from build123d import *

# Parameters (mm, degrees)
BOSS_EXTRUDE1_DEPTH             = 245
SKETCH6_R                       = 23.25
CUT_EXTRUDE1_DEPTH              = 3
F_6_5_6_5_DIAMETER_HOLE1_D      = 6.5
F_12_0_12_DIAMETER_HOLE1_REACH  = 253.446
F_12_0_12_DIAMETER_HOLE1_BORE_R = 6
M4_TAPPED_HOLE1_REACH           = 253.446
M4_TAPPED_HOLE1_BORE_R          = 1.65
CUT_EXTRUDE2_DEPTH              = 259.505319094
SKETCH12_R                      = 5
BOSS_EXTRUDE2_DEPTH             = 3
M5_TAPPED_HOLE1_D               = 4.2
M3_TAPPED_HOLE1_D               = 2.5
M3_TAPPED_HOLE1_DEPTH           = 3
CUT_EXTRUDE3_REACH              = 253.446
SKETCH17_R                      = 4


with BuildPart() as part:
    # Sketch1 → Boss-Extrude1 (new body)
    with BuildSketch(Plane.XY):
        with BuildLine():
            Line((-35, 20), (35, 20))
            ThreePointArc((35, 20), (38.535533906, 18.535533906), (40, 15))
            Line((40, 15), (40, -15))
            ThreePointArc((40, -15), (38.535533906, -18.535533906), (35, -20))
            Line((35, -20), (-35, -20))
            ThreePointArc((-35, -20), (-38.535533906, -18.535533906), (-40, -15))
            Line((-40, -15), (-40, 15))
            ThreePointArc((-40, 15), (-38.535533906, 18.535533906), (-35, 20))
        make_face()
        with BuildLine():
            Line((-37, 15), (-37, -15))
            ThreePointArc((-37, -15), (-36.414213562, -16.414213562), (-35, -17))
            Line((-35, -17), (35, -17))
            ThreePointArc((35, -17), (36.414213562, -16.414213562), (37, -15))
            Line((37, -15), (37, 15))
            ThreePointArc((37, 15), (36.414213562, 16.414213562), (35, 17))
            Line((35, 17), (-35, 17))
            ThreePointArc((-35, 17), (-36.414213562, 16.414213562), (-37, 15))
        make_face(mode=Mode.SUBTRACT)
    extrude(amount=BOSS_EXTRUDE1_DEPTH)

    # Sketch6 → Cut-Extrude1 (cut)
    with BuildSketch(Plane.XZ.offset(20)):
        with Locations(Location((0, 42, 0), (0, 0, 270))):
            Circle(SKETCH6_R)
    extrude(amount=-CUT_EXTRUDE1_DEPTH, mode=Mode.SUBTRACT)

    # Ø6.5 (6.5) Diameter Hole1 (through all)
    with Locations(Plane(origin=(0, 20, 0), x_dir=(1, 0, 0), z_dir=(0, 1, 0))):
        with Locations((-25, -17), (25, -17), (25, -67), (-25, -67)):
            Hole(F_6_5_6_5_DIAMETER_HOLE1_D / 2)

    # Ø12.0 (12) Diameter Hole1 bore → Ø12.0 (12) Diameter Hole1 (cut, up to next)
    with BuildSketch(Plane(origin=(0, 20, 0), x_dir=(1, 0, 0), z_dir=(0, 1, 0)), mode=Mode.PRIVATE) as f_12_0_12_diameter_hole1_sk1:
        with Locations((-25, -17)):
            Circle(F_12_0_12_DIAMETER_HOLE1_BORE_R)
    f_12_0_12_diameter_hole1_tool1 = extrude(f_12_0_12_diameter_hole1_sk1.sketch, amount=-F_12_0_12_DIAMETER_HOLE1_REACH, mode=Mode.PRIVATE) & part.part
    # Ø12.0 (12) Diameter Hole1 bore → Ø12.0 (12) Diameter Hole1 (cut, up to next)
    with BuildSketch(Plane(origin=(0, 20, 0), x_dir=(1, 0, 0), z_dir=(0, 1, 0)), mode=Mode.PRIVATE) as f_12_0_12_diameter_hole1_sk2:
        with Locations((25, -17)):
            Circle(F_12_0_12_DIAMETER_HOLE1_BORE_R)
    f_12_0_12_diameter_hole1_tool2 = extrude(f_12_0_12_diameter_hole1_sk2.sketch, amount=-F_12_0_12_DIAMETER_HOLE1_REACH, mode=Mode.PRIVATE) & part.part
    # Ø12.0 (12) Diameter Hole1 bore → Ø12.0 (12) Diameter Hole1 (cut, up to next)
    with BuildSketch(Plane(origin=(0, 20, 0), x_dir=(1, 0, 0), z_dir=(0, 1, 0)), mode=Mode.PRIVATE) as f_12_0_12_diameter_hole1_sk3:
        with Locations((25, -67)):
            Circle(F_12_0_12_DIAMETER_HOLE1_BORE_R)
    f_12_0_12_diameter_hole1_tool3 = extrude(f_12_0_12_diameter_hole1_sk3.sketch, amount=-F_12_0_12_DIAMETER_HOLE1_REACH, mode=Mode.PRIVATE) & part.part
    # Ø12.0 (12) Diameter Hole1 bore → Ø12.0 (12) Diameter Hole1 (cut, up to next)
    with BuildSketch(Plane(origin=(0, 20, 0), x_dir=(1, 0, 0), z_dir=(0, 1, 0)), mode=Mode.PRIVATE) as f_12_0_12_diameter_hole1_sk4:
        with Locations((-25, -67)):
            Circle(F_12_0_12_DIAMETER_HOLE1_BORE_R)
    f_12_0_12_diameter_hole1_tool4 = extrude(f_12_0_12_diameter_hole1_sk4.sketch, amount=-F_12_0_12_DIAMETER_HOLE1_REACH, mode=Mode.PRIVATE) & part.part
    add(f_12_0_12_diameter_hole1_tool1.solids().sort_by_distance((-25, 20, 17))[0], mode=Mode.SUBTRACT)
    add(f_12_0_12_diameter_hole1_tool2.solids().sort_by_distance((25, 20, 17))[0], mode=Mode.SUBTRACT)
    add(f_12_0_12_diameter_hole1_tool3.solids().sort_by_distance((25, 20, 67))[0], mode=Mode.SUBTRACT)
    add(f_12_0_12_diameter_hole1_tool4.solids().sort_by_distance((-25, 20, 67))[0], mode=Mode.SUBTRACT)

    # M4 Tapped Hole1 bore → M4 Tapped Hole1 (cut, up to next)
    with BuildSketch(Plane(origin=(0, 20, 0), x_dir=(1, 0, 0), z_dir=(0, 1, 0)), mode=Mode.PRIVATE) as m4_tapped_hole1_sk1:
        with Locations((-32.5, -9.5)):
            Circle(M4_TAPPED_HOLE1_BORE_R)
    m4_tapped_hole1_tool1 = extrude(m4_tapped_hole1_sk1.sketch, amount=-M4_TAPPED_HOLE1_REACH, mode=Mode.PRIVATE) & part.part
    # M4 Tapped Hole1 bore → M4 Tapped Hole1 (cut, up to next)
    with BuildSketch(Plane(origin=(0, 20, 0), x_dir=(1, 0, 0), z_dir=(0, 1, 0)), mode=Mode.PRIVATE) as m4_tapped_hole1_sk2:
        with Locations((32.5, -9.5)):
            Circle(M4_TAPPED_HOLE1_BORE_R)
    m4_tapped_hole1_tool2 = extrude(m4_tapped_hole1_sk2.sketch, amount=-M4_TAPPED_HOLE1_REACH, mode=Mode.PRIVATE) & part.part
    # M4 Tapped Hole1 bore → M4 Tapped Hole1 (cut, up to next)
    with BuildSketch(Plane(origin=(0, 20, 0), x_dir=(1, 0, 0), z_dir=(0, 1, 0)), mode=Mode.PRIVATE) as m4_tapped_hole1_sk3:
        with Locations((32.5, -74.5)):
            Circle(M4_TAPPED_HOLE1_BORE_R)
    m4_tapped_hole1_tool3 = extrude(m4_tapped_hole1_sk3.sketch, amount=-M4_TAPPED_HOLE1_REACH, mode=Mode.PRIVATE) & part.part
    # M4 Tapped Hole1 bore → M4 Tapped Hole1 (cut, up to next)
    with BuildSketch(Plane(origin=(0, 20, 0), x_dir=(1, 0, 0), z_dir=(0, 1, 0)), mode=Mode.PRIVATE) as m4_tapped_hole1_sk4:
        with Locations((-32.5, -74.5)):
            Circle(M4_TAPPED_HOLE1_BORE_R)
    m4_tapped_hole1_tool4 = extrude(m4_tapped_hole1_sk4.sketch, amount=-M4_TAPPED_HOLE1_REACH, mode=Mode.PRIVATE) & part.part
    add(m4_tapped_hole1_tool1.solids().sort_by_distance((-32.5, 20, 9.5))[0], mode=Mode.SUBTRACT)
    add(m4_tapped_hole1_tool2.solids().sort_by_distance((32.5, 20, 9.5))[0], mode=Mode.SUBTRACT)
    add(m4_tapped_hole1_tool3.solids().sort_by_distance((32.5, 20, 74.5))[0], mode=Mode.SUBTRACT)
    add(m4_tapped_hole1_tool4.solids().sort_by_distance((-32.5, 20, 74.5))[0], mode=Mode.SUBTRACT)

    # Sketch9 → Cut-Extrude2 (cut, through all)
    with BuildSketch(Plane(origin=(40, 0, 0), x_dir=(0, 0, -1), z_dir=(1, 0, 0))):
        Polygon((-245, 17), (-245, -20), (-211, -20), (-211, -17), align=None)
    extrude(amount=-CUT_EXTRUDE2_DEPTH, mode=Mode.SUBTRACT)

    # Sketch12 → Boss-Extrude2 (add)
    with BuildSketch(Plane.XZ.offset(-17)):
        with Locations((-28, 215)):
            Circle(SKETCH12_R)
        with Locations((-28, 235)):
            Circle(SKETCH12_R)
        with Locations((28, 215)):
            Circle(SKETCH12_R)
        with Locations((28, 235)):
            Circle(SKETCH12_R)
    extrude(amount=BOSS_EXTRUDE2_DEPTH)

    # M5 Tapped Hole1 (through all)
    with Locations(Plane(origin=(-35, 20, 20), x_dir=(1, 0, 0), z_dir=(0, 1, 0))):
        with Locations((7, -195), (7, -215), (63, -195), (63, -215)):
            Hole(M5_TAPPED_HOLE1_D / 2)

    # M3 Tapped Hole1
    with Locations(Plane(origin=(0, -20, 0), x_dir=(-1, 0, 0), z_dir=(0, -1, 0))):
        with Locations((26.5, -42), (-26.5, -42)):
            Hole(M3_TAPPED_HOLE1_D / 2, depth=M3_TAPPED_HOLE1_DEPTH)

    # Sketch17 → Cut-Extrude3 (cut, up to next)
    with BuildSketch(Plane(origin=(0, 20, 0), x_dir=(1, 0, 0), z_dir=(0, 1, 0)), mode=Mode.PRIVATE) as cut_extrude3_sk1:
        with Locations(Location((-26.5, -42, 0), (0, 0, 270))):
            Circle(SKETCH17_R)
    cut_extrude3_tool1 = extrude(cut_extrude3_sk1.sketch, amount=-CUT_EXTRUDE3_REACH, mode=Mode.PRIVATE) & part.part
    # Sketch17 → Cut-Extrude3 (cut, up to next)
    with BuildSketch(Plane(origin=(0, 20, 0), x_dir=(1, 0, 0), z_dir=(0, 1, 0)), mode=Mode.PRIVATE) as cut_extrude3_sk2:
        with Locations(Location((26.5, -42, 0), (0, 0, 270))):
            Circle(SKETCH17_R)
    cut_extrude3_tool2 = extrude(cut_extrude3_sk2.sketch, amount=-CUT_EXTRUDE3_REACH, mode=Mode.PRIVATE) & part.part
    add(cut_extrude3_tool1.solids().sort_by_distance((-26.5, 20, 42))[0], mode=Mode.SUBTRACT)
    add(cut_extrude3_tool2.solids().sort_by_distance((26.5, 20, 42))[0], mode=Mode.SUBTRACT)


solid = part.part
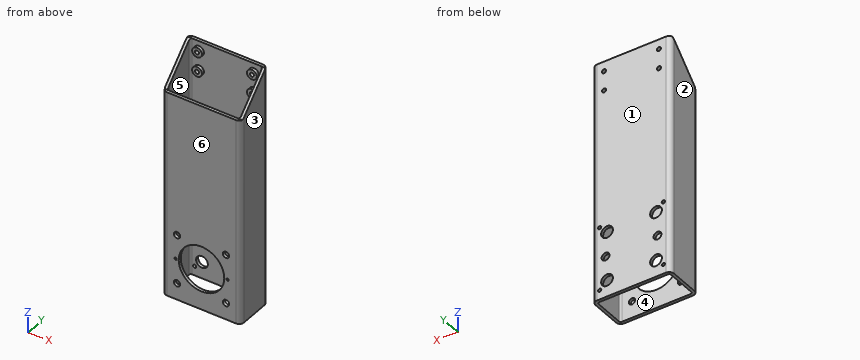
The listing builds one solid part. Answer for the finished solid, in the listing's coordinates (mm). Face numbers are marked on the shaded views. A direction names the side the tool comes from. Give positions to 0.01 mm unless a question says otherwise; leave off trailing zeros. Write each loop counter-clockwise with the first axis right and the second up, starting at its lowest first coordinate (ties: lowest second). Pieces come first, ordered by that corner, then holes.
Item 1: Section B-B, the plane z = 194.5 is taken. Write down the section's boundary in (x, y), plus the area to 3 significant figures.
Item 2: Section A-A, the plane y = -12 is taken. Write down the section's boundary in (x, z).
Item 3: Flat-ended cylindrical pins translate along their axes: P1, Ø1.5, axis at x = 30, y = -14.5, coming from the +Z side; P2, Ø2, axis at x = 32.5, z = 74.5, coming from the +Y side. Find the tip coordinate at first contact, or state that the pin passes through.
Item 4: Section C-C, the plane y = 4 is taken. Write down the section's boundary in (x, z).
Item 5: Section D-D, the plane x = -14.5 is taken. Write down the section's boundary in (y, z), plus the area to 3 significant figures.
Item 6: Determine the mould class of the marked faces 1, 2, 3 and 4 for opening direction X: released by +X, released by -X, zero draft, split by the parting line, or undercut.
Item 7: Which of the six approach directions +Z, -Z, +X, -X, +Y, -Y give full straight-line access (tool end or side, diameter ignored) to the marked faces 5 and 6?
Item 8: Find the intervals of material crossed by line 1 along X through (y, z) = (-7, 165); line 2 along Y through (x, z) = (23, 94); line 3 along Z through (x, y) = (25, -19.05), in increasing order.
Completed:
1. outline: (-40, -15) arc R5 ccw to (-35, -20) - (35, -20) arc R5 ccw to (40, -15) - (40, 15) arc R5 ccw to (35, 20) - (-35, 20) arc R5 ccw to (-40, 15) - close; hole (-37, -15) arc R2 ccw to (-35, -17) - (35, -17) arc R2 ccw to (37, -15) - (37, 15) arc R2 ccw to (35, 17) - (-35, 17) arc R2 ccw to (-37, 15) - close
1. area: 666 mm2
2. outline: (-40, 0) - (-37, 0) - (-37, 216) - (-40, 216) - close; (37, 0) - (40, 0) - (40, 216) - (37, 216) - close
3. P1: passes through
3. P2: stops at y = -17
4. outline: (-40, 0) - (-37, 0) - (-37, 232) - (-40, 232) - close; (37, 0) - (40, 0) - (40, 232) - (37, 232) - close
5. outline: (-20, 0) - (-17, 0) - (-17, 23.83) - (-20, 23.83) - close; (-20, 60.17) - (-17, 60.17) - (-17, 211) - (-20, 211) - close; (17, 0) - (20, 0) - (20, 245) - (17, 245) - close
5. area: 1,260 mm2
6. face 1: zero draft
6. face 2: released by -X
6. face 3: released by +X
6. face 4: undercut
7. face 5: +Z, -Z
7. face 6: +Z, -Z, +X, -X, -Y
8. line 1: x = -40 to -37, 37 to 40
8. line 2: y = -20 to -17, 17 to 20
8. line 3: z = 0 to 13.75, 20.25 to 63.75, 70.25 to 211
